Check sheet for the drawn part. Datum: minimum x, y, z corner. Units: mm. Round coordinates to 2 decimals unless told otherwise and drop trailing zeros. Write each loop counter-clockwise with the first axis right and the second up, starting at its lowest first coordinate (ties: lowest second). Pieces come first, ordered by that corner, then holes. Notation, with made-up numbers: (25, -20) -> (57, -20) arc R7 ccw to (57, -13) -> close; hole circle Ø2 at (-13.75, 79.5). An arc over 180 degrees is marked (long way). Use a Markdown table: item, result.
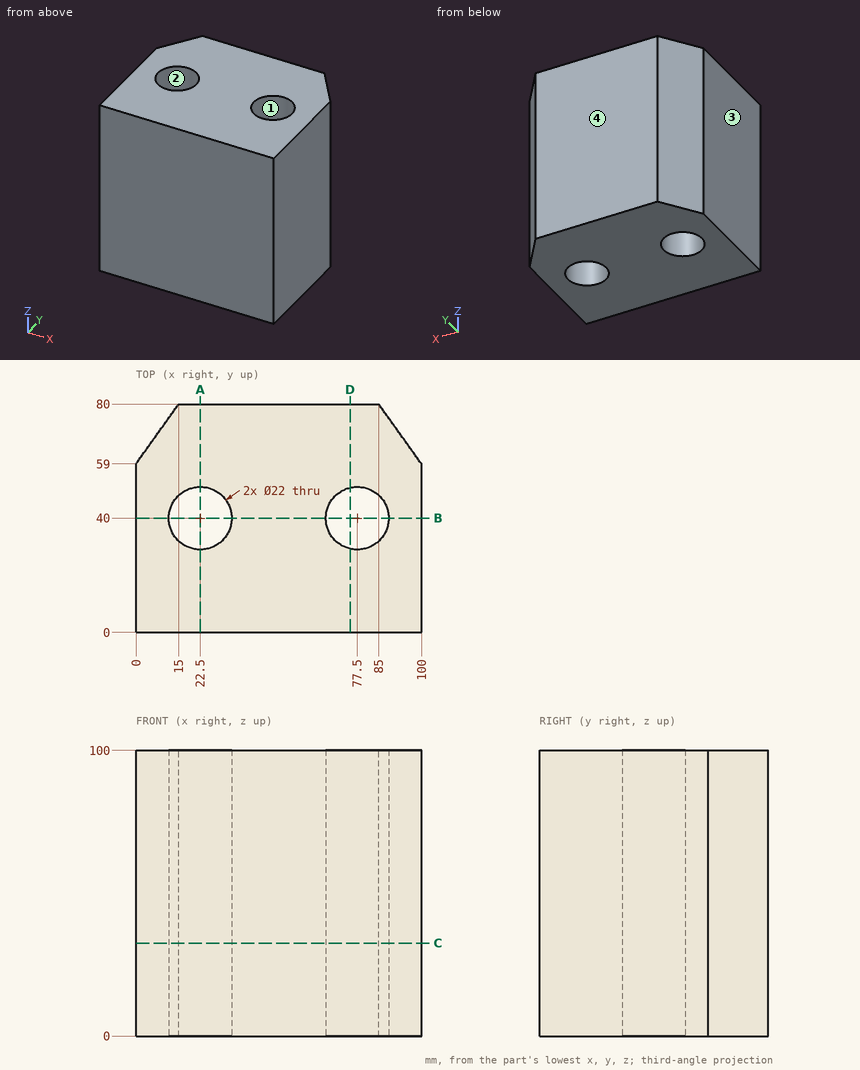
(1) Release check for a two-part mould opening along Y. For the marked faces 1, 2, 3 and 4 record: +Y half, -Y half, draft (parallel to the pull), parting line (faces both ways), or undercut.
A:
| item | result |
|---|---|
| face 1 | undercut |
| face 2 | undercut |
| face 3 | draft |
| face 4 | +Y half |
(2) Section check C-C on z = 32.5. Record the cut outline in (x, y), plus the area to 3 significant figures.
A:
| item | result |
|---|---|
| outline | (0, 0) -> (100, 0) -> (100, 59) -> (85, 80) -> (15, 80) -> (0, 59) -> close; hole circle Ø22 at (22.5, 40); hole circle Ø22 at (77.5, 40) |
| area | 6,920 mm2 |
(3) Section check B-B on y = 40. Record the cut outline in (x, z), plus the area to 3 significant figures.
A:
| item | result |
|---|---|
| outline | (0, 0) -> (11.5, 0) -> (11.5, 100) -> (0, 100) -> close; (33.5, 0) -> (66.5, 0) -> (66.5, 100) -> (33.5, 100) -> close; (88.5, 0) -> (100, 0) -> (100, 100) -> (88.5, 100) -> close |
| area | 5,600 mm2 |
(4) Gauge pin test, flat end, axial feed: pin 1 Ø17.5 at (x, y) = (77.5, 40) entering from -Z. Record the tip position at first contact, or that the pin passes through.
A:
| item | result |
|---|---|
| pin 1 | passes through |
(5) Section check D-D on x = 75. Record the cut outline in (y, z).
A:
| item | result |
|---|---|
| outline | (0, 0) -> (29.29, 0) -> (29.29, 100) -> (0, 100) -> close; (50.71, 0) -> (80, 0) -> (80, 100) -> (50.71, 100) -> close |
(6) Thickness scan on line 1 (Y direction, x = 22, z = 68); line 2 (X direction, y = 50, z = 45); line 3 (Y direction, x = 70, z = 20). Record the ranges inside material, lowest first.
A:
| item | result |
|---|---|
| line 1 | y = 0 to 29.01, 50.99 to 80 |
| line 2 | x = 0 to 17.92, 27.08 to 72.92, 82.08 to 100 |
| line 3 | y = 0 to 31.95, 48.05 to 80 |
(7) Section check A-A on x = 22.5. Record the cut outline in (y, z), plus the area to 3 significant figures.
A:
| item | result |
|---|---|
| outline | (0, 0) -> (29, 0) -> (29, 100) -> (0, 100) -> close; (51, 0) -> (80, 0) -> (80, 100) -> (51, 100) -> close |
| area | 5,800 mm2 |
